```python
from build123d import *

# Parameters (mm, degrees)
SKETCH1_W           = 220
SKETCH1_H           = 140
SKETCH1_R           = 7
BOSS_EXTRUDE1_DEPTH = 10
FILLET1_R           = 10


with BuildPart() as part:
    # Sketch1 → Boss-Extrude1 (new body)
    with BuildSketch(Plane.XY):
        Rectangle(SKETCH1_W, SKETCH1_H)
        with Locations((-95, 0)):
            Circle(SKETCH1_R, mode=Mode.SUBTRACT)
        with Locations((95, 0)):
            Circle(SKETCH1_R, mode=Mode.SUBTRACT)
    extrude(amount=BOSS_EXTRUDE1_DEPTH)

    # Fillet1
    fillet1_edges = [part.edges().sort_by_distance(p)[0] for p in [
        (-110, 70, 5),
        (110, 70, 5),
        (110, -70, 5),
        (-110, -70, 5),
    ]]
    fillet(fillet1_edges, radius=FILLET1_R)


solid = part.part
```
For this review, take the finished solid that the model builds, in its own axes (mm). Round coordinates to 2 decimals unless told otherwise and drop trailing zeros. Write each loop counter-clockwise with the first axis right and the second up, starting at its lowest first coordinate (ties: lowest second). Pieces come first, ordered by that corner, then holes. Notation, with made-up numbers: (69.25, -3) - (96.25, -3) arc R14 cw to (96.25, 7) - close; hole circle Ø6 at (-15, 53.5). An arc over 180 degrees is marked (long way). Answer as CSV lines item,"result". Start each with the question number.
(1) For line 1 (Y direction, x = -95, z = 7.75); line 2 (X direction, y = -3, z = 3.75); line 3 (X direction, y = -5.5, z = 3), list the stretches that pass through material, from the lowest coordinate up.
(2) Add section A-A, the plane x = 95. State the section outline as (y, z) points.
(3) Mouldability with a two-part tool opening along X and no side actions: class faces 1 (the cylindrical face through (106.99, 67.15, 5.07)), 2 (the cylindrical face through (-107.15, -66.99, 5.07)), 3 (the flat face through (-2, 1, 10)), 4 (the cylindrical face through (-102, 0, 5)) as +X half, -X half, draft (parallel to the pull), parting line (faces both ways), or undercut.
(4) Add section C-C, the plane x = -90.5. State the section outline as (y, z) points, plus the area to 3 significant figures.
(5) Add section B-B, the plane y = 0. State the section outline as (x, z) points.
From the geometry:
1,line 1,"y = -70 to -7, 7 to 70"
1,line 2,"x = -110 to -101.32, -88.68 to 88.68, 101.32 to 110"
1,line 3,"x = -110 to -99.33, -90.67 to 90.67, 99.33 to 110"
2,outline,"(-70, 0) - (-7, 0) - (-7, 10) - (-70, 10) - close; (7, 0) - (70, 0) - (70, 10) - (7, 10) - close"
3,face 1,"+X half"
3,face 2,"-X half"
3,face 3,"draft"
3,face 4,"undercut"
4,outline,"(-70, 0) - (-5.36, 0) - (-5.36, 10) - (-70, 10) - close; (5.36, 0) - (70, 0) - (70, 10) - (5.36, 10) - close"
4,area,"1,290 mm²"
5,outline,"(-110, 0) - (-102, 0) - (-102, 10) - (-110, 10) - close; (-88, 0) - (88, 0) - (88, 10) - (-88, 10) - close; (102, 0) - (110, 0) - (110, 10) - (102, 10) - close"
